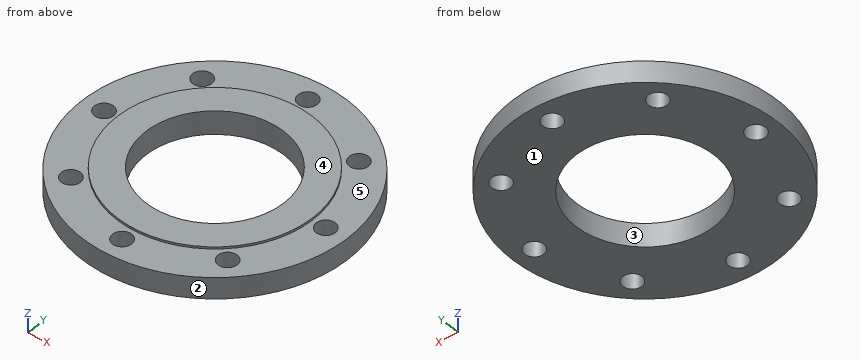
```python
from build123d import *

# Parameters (mm, degrees)
SKETCH1_R           = 125
SKETCH1_R_2         = 65
SKETCH1_R_3         = 9
BOSS_EXTRUDE1_DEPTH = 20
SKETCH2_R           = 92
SKETCH2_R_2         = 65
BOSS_EXTRUDE2_DEPTH = 2


with BuildPart() as part:
    # Sketch1 → Boss-Extrude1 (new body)
    with BuildSketch(Plane.XY):
        Circle(SKETCH1_R)
        Circle(SKETCH1_R_2, mode=Mode.SUBTRACT)
        with Locations((0, 105)):
            Circle(SKETCH1_R_3, mode=Mode.SUBTRACT)
        with Locations((74.246212025, 74.246212025)):
            Circle(SKETCH1_R_3, mode=Mode.SUBTRACT)
        with Locations((105, 0)):
            Circle(SKETCH1_R_3, mode=Mode.SUBTRACT)
        with Locations((74.246212025, -74.246212025)):
            Circle(SKETCH1_R_3, mode=Mode.SUBTRACT)
        with Locations((0, -105)):
            Circle(SKETCH1_R_3, mode=Mode.SUBTRACT)
        with Locations((-74.246212025, -74.246212025)):
            Circle(SKETCH1_R_3, mode=Mode.SUBTRACT)
        with Locations((-105, 0)):
            Circle(SKETCH1_R_3, mode=Mode.SUBTRACT)
        with Locations((-74.246212025, 74.246212025)):
            Circle(SKETCH1_R_3, mode=Mode.SUBTRACT)
    extrude(amount=BOSS_EXTRUDE1_DEPTH)

    # Sketch2 → Boss-Extrude2 (add)
    with BuildSketch(Plane.XY.offset(20)):
        Circle(SKETCH2_R)
        Circle(SKETCH2_R_2, mode=Mode.SUBTRACT)
    extrude(amount=BOSS_EXTRUDE2_DEPTH)


solid = part.part
```
For this review, take the finished solid that the model builds, in its own axes (mm). Face numbers are marked on the shaded views. A direction names the side the tool comes from. Round coordinates to 2 decimals unless told otherwise and drop trailing zeros. Loops run counter-clockwise (first coordinate to the right, second up) from the corner with the lowest first, then second, coordinate; pieces in that order, holes last.
Q1. Add section A-A on x = 0. Write out the cut boundary in (y, z).
Result sheet:
outline: (-125, 0) - (-114, 0) - (-114, 20) - (-125, 20) - close; (-96, 0) - (-65, 0) - (-65, 22) - (-92, 22) - (-92, 20) - (-96, 20) - close; (65, 0) - (96, 0) - (96, 20) - (92, 20) - (92, 22) - (65, 22) - close; (114, 0) - (125, 0) - (125, 20) - (114, 20) - close
Q2. Add section D-D on x = 105. Write out the cut boundary in (y, z).
Result sheet:
outline: (-67.82, 0) - (-9, 0) - (-9, 20) - (-67.82, 20) - close; (9, 0) - (67.82, 0) - (67.82, 20) - (9, 20) - close
Q3. Insertion check: pin 1 Ø2 at (y, z) = (-5.5, 13) entering from -X; pin 2 Ø20.5 at (x, y) = (-105, 0) entering from +Z; pin 3 Ø10 at (x, z) = (-91.5, 6.5) entering from +Y. Each pin has a flat end and moves straight along its axis. Give the tip position at first contact, or say it passes through.
Result sheet:
pin 1: stops at x = -124.92
pin 2: stops at z = 20
pin 3: stops at y = 90.24
Q4. Add section C-C on y = 32. Write out the cut boundary in (x, z).
Result sheet:
outline: (-120.83, 0) - (-56.58, 0) - (-56.58, 22) - (-86.26, 22) - (-86.26, 20) - (-120.83, 20) - close; (56.58, 0) - (120.83, 0) - (120.83, 20) - (86.26, 20) - (86.26, 22) - (56.58, 22) - close
Q5. Machinability: for the marked faces 4 and 5, which of the approach directions +Z, -Z, +X, -X, +Y, -Y give a long, thin tool a straight path to every point of the face, cutting with its end or side? Answer none if there is none.
Result sheet:
face 4: +Z, +X, -X, +Y, -Y
face 5: +Z
Q6. To check wall thickness, follow line 1 along Y through (x, z) = (0, 11.5); line 2 along Y through (x, z) = (3, 13); line 3 along Y through (x, z) = (78, 5.5). State the ranges of each line that lie inside material, in increasing order.
Result sheet:
line 1: y = -125 to -114, -96 to -65, 65 to 96, 114 to 125
line 2: y = -124.96 to -113.49, -96.51 to -64.93, 64.93 to 96.51, 113.49 to 124.96
line 3: y = -97.68 to -82.43, -66.07 to 66.07, 82.43 to 97.68
Q7. Mouldability with a two-part tool opening along X and no side actions: class the marked faces 1, 2 and 3 as +X half, -X half, draft (parallel to the pull), parting line (faces both ways), or undercut.
Result sheet:
face 1: draft
face 2: parting line
face 3: undercut
